Verification items for the finished model (mm, model axes). A direction names the side the tool comes from. Give positions to 0.01 mm unless a question says otherwise; leave off trailing zeros. Order: outer loops, then holes, each group sorted by start corner. A loop starts at its lowest first (then second) coordinate and runs counter-clockwise, first axis right, second up. Notation, with made-up numbers: (-37, -12) -> (-13, -12) arc R18 ccw to (-13, 9) -> close; hole circle Ø7 at (44.5, 7.25). An arc over 180 degrees is marked (long way). Return JSON: item names as keys, results as strings. Group by question number.
(1) Cross-section at D-D on x = 1.5. Enter the section's corners in (y, z).
(2) Release check for a two-part mould opening along Y. For faces 3 (the face through (-1, -7.1, 0.5)), 4 (the face through (-3.595, -7.002, 0.542)), 5 (the face through (4.8, -6.32, 0.54)) record: pulls with the +Y half, pulls with the -Y half, needs draft (parallel to the pull), parting line crosses it, or undercut.
(3) Tool access check on faces 1 (the face through (1, -7.1, 0.5)), 2 (the face through (2.794, -8.345, 0.542)). Record the directions out of +Z, -Z, +X, -X, +Y, -Y that give a thin tool (end or side, any length) a straight path to the whole face; none if there is none.
(4) Thickness scan on line 1 along Y through (x, z) = (-3, 0.6); line 2 along Y through (x, z) = (2.5, 0.75); line 3 along X through (y, z) = (5, 0.5). Record the ranges inside material, lowest first.
(5) Cross-section at B-B on x = 3. Enter the section's corners in (y, z), then the cut area to 3 significant figures.
(6) Cross-section at C-C on z = 0.8. Enter the section's corners in (x, y), then the cut area to 3 significant figures.
(7) Depth check by flat-ended pin: pin 1 Ø0.6 at (y, z) = (-8, 0.5) entering from +X. Enter the tip coordinate at first touch or a pass-through.
(8) Cross-section at A-A on y = -2.75. Enter the section's corners in (x, z).
from build123d import *

# Parameters (mm, degrees)
SKETCH1_R           = 0.75
BOSS_EXTRUDE1_DEPTH = 1.1


with BuildPart() as part:
    # Sketch1 → Boss-Extrude1 (new body)
    with BuildSketch(Plane.XY):
        with BuildLine():
            Line((1, -5.408326913), (1, -6.326068688))
            Line((1, -6.326068688), (1, -7.130217388))
            Line((1, -7.130217388), (1, -8.742997198))
            ThreePointArc((1, -8.742997198), (2.818656417, -8.336376671), (4.510908199, -7.555905454))
            ThreePointArc((4.510908199, -7.555905454), (4.573051873, -7.497695365), (4.605349108, -7.418909965))
            Line((4.605349108, -7.418909965), (5, -5.180733539))
            Line((5, -5.180733539), (5.160454845, -4.028284746))
            ThreePointArc((5.160454845, -4.028284746), (0, 7.2), (-5.160454845, -4.028284746))
            Line((-5.160454845, -4.028284746), (-5, -5.180733539))
            Line((-5, -5.180733539), (-4.605349108, -7.418909965))
            ThreePointArc((-4.605349108, -7.418909965), (-4.573051873, -7.497695365), (-4.510908199, -7.555905454))
            ThreePointArc((-4.510908199, -7.555905454), (-2.818656417, -8.336376671), (-1, -8.742997198))
            Line((-1, -8.742997198), (-1, -7.130217388))
            Line((-1, -7.130217388), (-1, -5.408326913))
            ThreePointArc((-1, -5.408326913), (0, 5.5), (1, -5.408326913))
        make_face()
        with Locations((-3, -6.545227269)):
            Circle(SKETCH1_R, mode=Mode.SUBTRACT)
        with Locations((3, -6.545227269)):
            Circle(SKETCH1_R, mode=Mode.SUBTRACT)
    extrude(amount=BOSS_EXTRUDE1_DEPTH)


solid = part.part
Verdict:
{
 "1": {"outline": "(-8.67, 0) -> (-5.29, 0) -> (-5.29, 1.1) -> (-8.67, 1.1) -> close; (5.29, 0) -> (7.03, 0) -> (7.03, 1.1) -> (5.29, 1.1) -> close"},
 "2": {"face 3": "needs draft", "face 4": "undercut", "face 5": "pulls with the -Y half"},
 "3": {"face 1": "+Z, -Z, -Y", "face 2": "+Z, -Z, +X, -Y"},
 "4": {"line 1": "-8.27 to -7.3, -5.8 to -4.61, 4.61 to 6.5", "line 2": "-8.44 to -7.1, -5.99 to -4.9, 4.9 to 6.72", "line 3": "-5.01 to -2.29, 2.29 to 5.01"},
 "5": {"outline": "(-8.27, 0) -> (-7.3, 0) -> (-7.3, 1.1) -> (-8.27, 1.1) -> close; (-5.8, 0) -> (-4.61, 0) -> (-4.61, 1.1) -> (-5.8, 1.1) -> close; (4.61, 0) -> (6.5, 0) -> (6.5, 1.1) -> (4.61, 1.1) -> close", "area": "4.46 mm²"},
 "6": {"outline": "(-5.16, -4.03) -> (-5, -5.18) -> (-4.61, -7.42) arc R0.2 ccw to (-4.51, -7.56) arc R8.8 ccw to (-1, -8.74) -> (-1, -5.41) arc R5.5 cw (long way) to (1, -5.41) -> (1, -8.74) arc R8.8 ccw to (4.51, -7.56) arc R0.2 ccw to (4.61, -7.42) -> (5, -5.18) -> (5.16, -4.03) arc R6.8 ccw (long way) to start; hole circle Ø1.5 at (-3, -6.55); hole circle Ø1.5 at (3, -6.55)", "area": "65.1 mm²"},
 "7": {"pin 1": "x = 4.26"},
 "8": {"outline": "(-6.03, 0) -> (-4.76, 0) -> (-4.76, 1.1) -> (-6.03, 1.1) -> close; (4.76, 0) -> (6.03, 0) -> (6.03, 1.1) -> (4.76, 1.1) -> close"}
}
